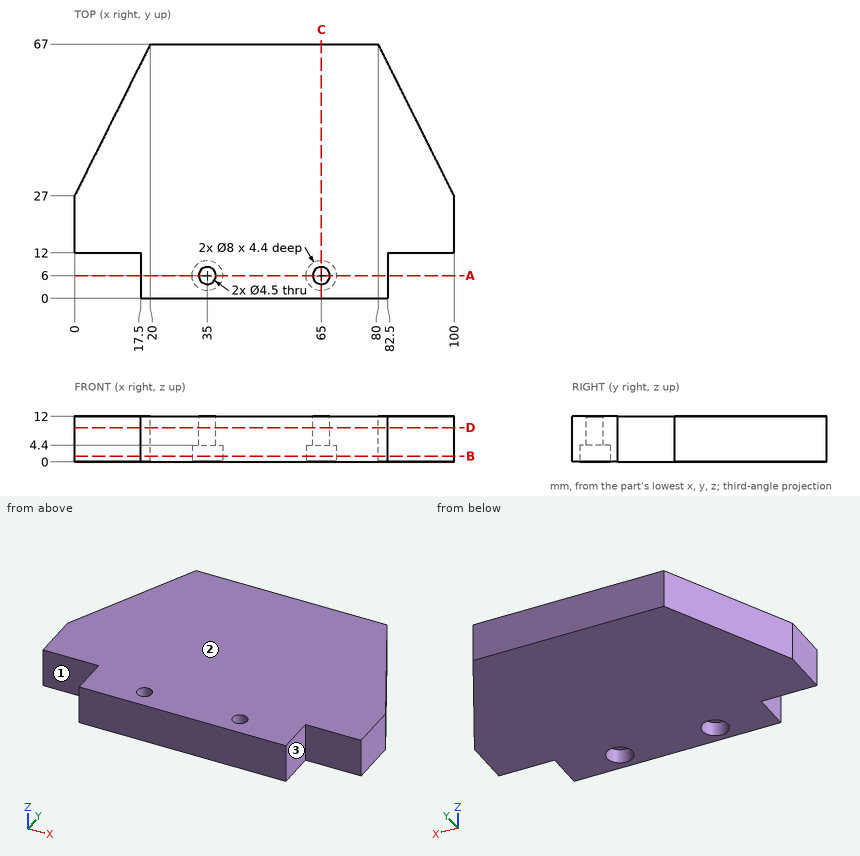
Study the drawing (mm; zero at the part's minimum x, y, z) and answer. A direction names the side the tool comes from. Give positions to 0.01 mm unless a question says otherwise; leave off trailing zeros. Write each loop counter-clockwise with the first axis right and the second up, starting at its lowest first coordinate (ties: lowest second). Pieces come first, ordered by that corner, then holes. Notation, with made-up numbers: (40, 3) - (83, 3) arc R15 cw to (83, 30) - close; hole circle Ø5 at (-17, 23). An arc over 180 degrees is marked (long way). Use a Markdown table: item, result.
1. Section C-C on x = 65 is taken. Write down the section's boundary in (y, z), plus the area to 3 significant figures.
Values follow:
| item | result |
|---|---|
| outline | (0, 0) - (2, 0) - (2, 4.4) - (3.75, 4.4) - (3.75, 12) - (0, 12) - close; (8.25, 4.4) - (10, 4.4) - (10, 0) - (67, 0) - (67, 12) - (8.25, 12) - close |
| area | 735 mm² |
2. A tool of negligible diameter and unlimited length cuts with its end or side. For the marked faces 1, 2 and 3, from which of +Z, -Z, +X, -X, +Y, -Y can it reach the whole face along a straight path? Write none if from no direction.
Values follow:
| item | result |
|---|---|
| face 1 | +Z, -Z, -X, -Y |
| face 2 | +Z, +X, -X, +Y, -Y |
| face 3 | +Z, -Z, +X, -Y |
3. Section B-B on z = 1.5 is taken. Write down the section's boundary in (x, y), plus the area to 3 significant figures.
Values follow:
| item | result |
|---|---|
| outline | (0, 12) - (17.5, 12) - (17.5, 0) - (82.5, 0) - (82.5, 12) - (100, 12) - (100, 27) - (80, 67) - (20, 67) - (0, 27) - close; hole circle Ø8 at (35, 6); hole circle Ø8 at (65, 6) |
| area | 5,380 mm² |
4. Each of these flat-tipped pins is pushed along its axis until it touches: P1, Ø5, axis at x = 65, y = 6, coming from the -Z side; P2, Ø3.5, axis at y = 6, z = 6.5, coming from the +X side; P3, Ø3, axis at x = 51.5, y = 57, coming from the -Z side; P4, Ø3, axis at x = 18, z = 7.5, coming from the +Y side. Where does it stop, or does it pass through?
Values follow:
| item | result |
|---|---|
| P1 | stops at z = 4.4 |
| P2 | stops at x = 82.5 |
| P3 | stops at z = 0 |
| P4 | stops at y = 66 |
5. Section A-A on y = 6 is taken. Write down the section's boundary in (x, z).
Values follow:
| item | result |
|---|---|
| outline | (17.5, 0) - (31, 0) - (31, 4.4) - (32.75, 4.4) - (32.75, 12) - (17.5, 12) - close; (37.25, 4.4) - (39, 4.4) - (39, 0) - (61, 0) - (61, 4.4) - (62.75, 4.4) - (62.75, 12) - (37.25, 12) - close; (67.25, 4.4) - (69, 4.4) - (69, 0) - (82.5, 0) - (82.5, 12) - (67.25, 12) - close |
6. Section D-D on z = 9 is taken. Write down the section's boundary in (x, y), plus the area to 3 significant figures.
Values follow:
| item | result |
|---|---|
| outline | (0, 12) - (17.5, 12) - (17.5, 0) - (82.5, 0) - (82.5, 12) - (100, 12) - (100, 27) - (80, 67) - (20, 67) - (0, 27) - close; hole circle Ø4.5 at (35, 6); hole circle Ø4.5 at (65, 6) |
| area | 5,450 mm² |
7. Find the intervals of material crossed by probe 1 along Y at (x, z) = (65, 10); probe 2 along X at (y, z) = (10, 7.25); probe 3 along Y at (x, z) = (63, 5.25), in increasing order. Write a range as from..to.
Values follow:
| item | result |
|---|---|
| probe 1 | y = 0..3.75, 8.25..67 |
| probe 2 | x = 17.5..82.5 |
| probe 3 | y = 0..4.97, 7.03..67 |
